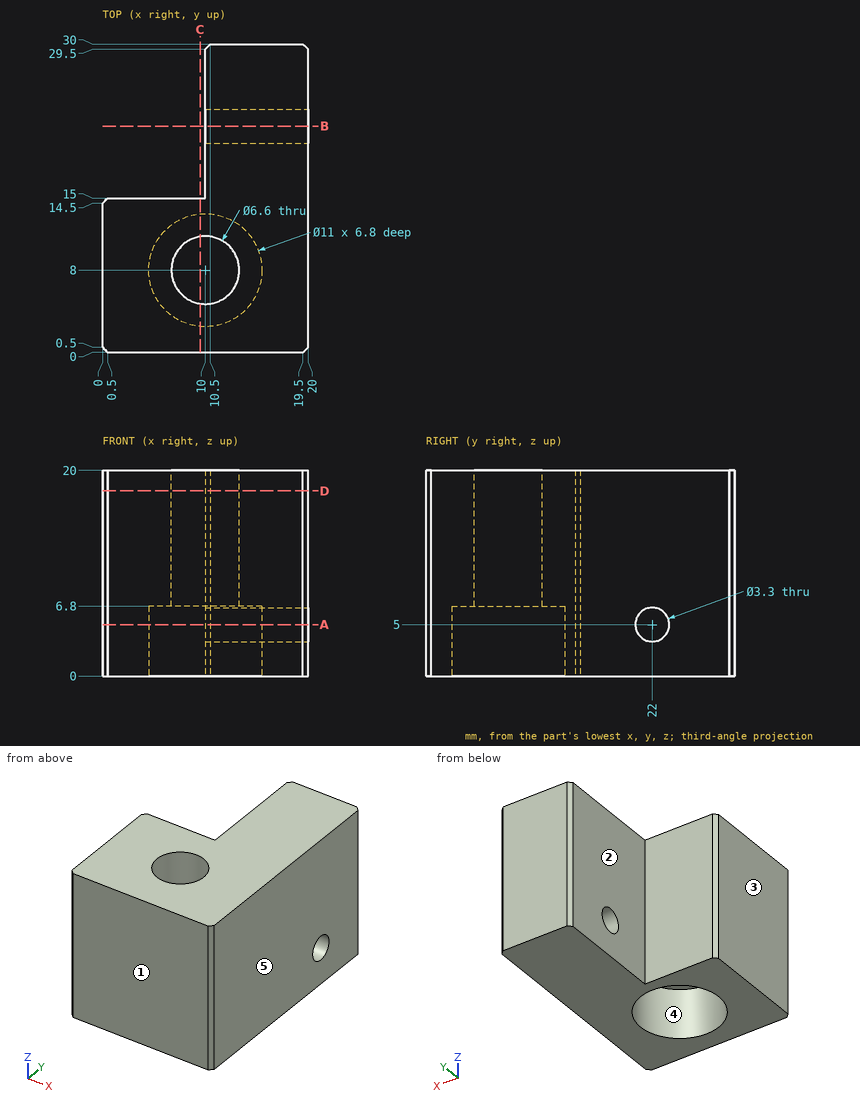
Could you check a few things on this drawing? It's one solid part, dimensions in mm from its lowest x, y, z. A direction names the side the tool comes from. Round coordinates to 2 decimals unless told otherwise and drop trailing zeros. Order: outer loops, then holes, each group sorted by start corner. A loop starts at its lowest first (then second) coordinate and runs counter-clockwise, first axis right, second up. Notation, with made-up numbers: M -40,19.25 L 4,19.25 A28 ccw 4,58.25 Z; hole C -4.75,-13 d8. An arc over 180 degrees is marked long. Return JSON: item names as keys, results as strings. Group by question number.
1. If we section it at B-B on y = 22: List the corners of the cut face in (x, z) for me.
2. On a 3-axis mill with a long thin cutter (end or side, diameter ignored), from which of +Z, -Z, +X, -X, +Y, -Y can I reach the whole of each face in a straight line? I mean the marked faces 1 and 2. Say none if no direction works.
3. If we mould it in two halves opening along X, with no side actions, what happens to the marked faces 3, 4 and 5? For each: pulls with the +X half, pulls with the -X half, needs draft (parallel to the pull), parting line crosses it, or undercut.
4. If we section it at C-C on x = 9.5: List the corners of the cut face in (y, z) for me, then the cut area to 3 significant figures.
5. Please list where these lines run through material, in increasing order: probe 1 along Y at (x, z) = (18, 5); probe 2 along Y at (x, z) = (13.75, 5); probe 3 along X at (y, z) = (6.5, 12.5).
6. I'm going to push flat-ended pins straight in: pin 1 Ø2 at (y, z) = (21.5, 7.5) entering from -X; pin 2 Ø10.5 at (x, z) = (3, 8.5) entering from +Y. Where does each tip first touch, or does it pass through?
7. If we section it at A-A on z = 5: List the corners of the cut face in (x, y) for me, then the cut area to 3 significant figures.
8. If we section it at D-D on z = 18: List the corners of the cut face in (x, y) for me, then the cut area to 3 significant figures.
Reply:
{
 "1": {"outline": "M 10,0 L 20,0 L 20,3.35 L 10,3.35 Z; M 10,6.65 L 20,6.65 L 20,20 L 10,20 Z"},
 "2": {"face 1": "+Z, -Z, +X, -X, -Y", "face 2": "+Z, -Z, -X, +Y"},
 "3": {"face 3": "pulls with the -X half", "face 4": "undercut", "face 5": "pulls with the +X half"},
 "4": {"outline": "M 0,0 L 2.52,0 L 2.52,6.8 L 4.74,6.8 L 4.74,20 L 0,20 Z; M 11.26,6.8 L 13.48,6.8 L 13.48,0 L 15,0 L 15,20 L 11.26,20 Z", "area": "139 mm^2"},
 "5": {"probe 1": "0 to 20.35, 23.65 to 30", "probe 2": "0 to 3.98, 12.02 to 20.35, 23.65 to 30", "probe 3": "0 to 7.06, 12.94 to 20"},
 "6": {"pin 1": "x = 10", "pin 2": "y = 15"},
 "7": {"outline": "M 0,0.5 L 0.5,0 L 19.5,0 L 20,0.5 L 20,20.35 L 10,20.35 L 10,15 L 0.5,15 L 0,14.5 Z; M 10,23.65 L 20,23.65 L 20,29.5 L 19.5,30 L 10.5,30 L 10,29.5 Z; hole C 10,8 d11", "area": "321 mm^2"},
 "8": {"outline": "M 0,0.5 L 0.5,0 L 19.5,0 L 20,0.5 L 20,29.5 L 19.5,30 L 10.5,30 L 10,29.5 L 10,15 L 0.5,15 L 0,14.5 Z; hole C 10,8 d6.6", "area": "415 mm^2"}
}
